from build123d import *

# Parameters (mm, degrees)
SKETCH1_R  = 1
BODY_DEPTH = 1.2


with BuildPart() as part:
    # Sketch1 → Body (new body)
    with BuildSketch(Plane.XY):
        with BuildLine():
            Line((5.186595963, -12.521550316), (6.142069089, -14.828266497))
            ThreePointArc((6.142069089, -14.828266497), (0, 16.05), (-6.142069089, -14.828266497))
            Line((-6.142069089, -14.828266497), (-5.186595963, -12.521550316))
            ThreePointArc((-5.186595963, -12.521550316), (-5.851927185, -10.143153881), (-8.32029392, -10.224399796))
            ThreePointArc((-8.32029392, -10.224399796), (-9.164022184, -10.503157731), (-9.968180846, -10.125120408))
            ThreePointArc((-9.968180846, -10.125120408), (0, 12.85), (9.968180846, -10.125120408))
            ThreePointArc((9.968180846, -10.125120408), (9.164022184, -10.503157731), (8.32029392, -10.224399796))
            ThreePointArc((8.32029392, -10.224399796), (5.851927185, -10.143153881), (5.186595963, -12.521550316))
        make_face()
        with Locations(Location((7.034355028, -11.756183451, 0), (0, 0, 180))):
            Circle(SKETCH1_R, mode=Mode.SUBTRACT)
        with Locations((-7.034355028, -11.756183451)):
            Circle(SKETCH1_R, mode=Mode.SUBTRACT)
    extrude(amount=-BODY_DEPTH)


solid = part.part
Check sheet for the modelled part. Datum: model origin and axes. Units: mm. A direction names the side the tool comes from. Round coordinates to 2 decimals unless told otherwise and drop trailing zeros. Order: outer loops, then holes, each group sorted by start corner. A loop starts at its lowest first (then second) coordinate and runs counter-clockwise, first axis right, second up.
(1) Cross-section at D-D, the plane x = 0. Enter the section's corners in (y, z).
(2) Go/stop test with a flat-tipped pin: P1, Ø1.2, axis at x = -7.03, y = -11.76, coming from the -Z side. Record where the tip stops, or that it passes through.
(3) Cross-section at C-C, the plane z = -0.7. Enter the section's corners in (x, y), and give its area (3 significant figures).
(4) Draft check along X on faces 1 (the cylindrical face through (0.62, 16.04, -0.59)), 2 (the flat face through (5.66, -13.66, -0.59)), 3 (the cylindrical face through (-8.033, -11.712, -0.592)), 4 (the flat face through (1, 13, 0)). Enter one of: pulls with the +X half, pulls with the -X half, needs draft (parallel to the pull), parting line crosses it, or undercut.
(5) Cross-section at A-A, the plane y = 0. Enter the section's corners in (x, z), and give its area (3 significant figures).
(6) Cross-section at B-B, the plane x = 9.5. Enter the section's corners in (y, z), and give its area (4 significant figures).
(7) Access from +Z, -Z, +X, -X, +Y, -Y to the whole of each face (thin tool, end or side, straight path). Record for faces 5 (the cylindrical face through (9.2, -10.5, -0.6)), 6 (the flat face through (-5.67, -13.69, -0.59)), 7 (the flat face through (1, 13, -1.2)).
(8) Scan lines: probe 1 along X at (y, z) = (-10, -0.5); probe 2 along X at (y, z) = (-0.5, -0.2); probe 3 along Y at (x, z) = (5.5, -0.2). Record each from-to range of solid material in increasing order.
Check sheet entries:
1. outline: (12.85, -1.2) - (16.05, -1.2) - (16.05, 0) - (12.85, 0) - close
2. P1: passes through
3. outline: (-9.97, -10.13) arc R13.65 cw (long way) to (9.97, -10.13) arc R1.2 cw to (8.32, -10.22) arc R2 ccw to (5.19, -12.52) - (6.14, -14.83) arc R16.05 ccw (long way) to (-6.14, -14.83) - (-5.19, -12.52) arc R2 ccw to (-8.32, -10.22) arc R1.2 cw to start; hole circle Ø2 at (-7.03, -11.76); hole circle Ø2 at (7.03, -11.76)
3. area: 216 mm2
4. face 1: parting line crosses it
4. face 2: undercut
4. face 3: undercut
4. face 4: needs draft
5. outline: (-16.05, -1.2) - (-13.63, -1.2) - (-13.63, 0) - (-16.05, 0) - close; (13.63, -1.2) - (16.05, -1.2) - (16.05, 0) - (13.63, 0) - close
5. area: 5.82 mm2
6. outline: (-12.94, -1.2) - (-10.43, -1.2) - (-10.43, 0) - (-12.94, 0) - close; (9, -1.2) - (12.94, -1.2) - (12.94, 0) - (9, 0) - close
6. area: 7.725 mm2
7. face 5: +Z, -Z
7. face 6: +Z, -Z, -Y
7. face 7: -Z, +X, -X, +Y, -Y
8. probe 1: x = -12.55 to -10.08, -7.99 to -6.08, 6.08 to 7.99, 10.08 to 12.55
8. probe 2: x = -16.04 to -13.65, 13.65 to 16.04
8. probe 3: y = -13.28 to -10.47, 11.69 to 15.08
